Source: CAD feature listing. Evaluate the final solid. Frame: model axes, mm. Coordinates: 2 decimals unless noted, no trailing zeros. Order: outer loops, then holes, each group sorted by start corner. A loop starts at its lowest first (then second) coordinate and runs counter-clockwise, first axis right, second up.
```python
from build123d import *

# Parameters (mm, degrees)
SKETCH_1_R      = 20
EXTRUDE_1_DEPTH = 44.4
SKETCH_2_W      = 2.53960462
SKETCH_2_H      = 1.7


with BuildPart() as part:
    # 草图1 → 凸台-拉伸1 (new body)
    with BuildSketch(Plane(origin=(0, 0, 0), x_dir=(1, 0, 0), z_dir=(0, 1, 0))):
        with Locations(Location((0, 0, 0), (0, 0, 270))):
            Circle(SKETCH_1_R)
    extrude(amount=EXTRUDE_1_DEPTH)

    # 草图2 → 切除-旋转1 (revolve, cut)
    with BuildSketch(Plane.XY, mode=Mode.PRIVATE) as cut_revolve_1_sk:
        with Locations((-20.01980231, 3.85)):
            Rectangle(SKETCH_2_W, SKETCH_2_H)
    cut_revolve_1 = revolve(cut_revolve_1_sk.sketch.rotate(Axis((0, 44.4, 0), (0, -1, 0)), 270), axis=Axis((0, 44.4, 0), (0, -1, 0)), mode=Mode.SUBTRACT)

    # 镜向1: 切除-旋转1 across plane
    add(cut_revolve_1.mirror(Plane(origin=(0, 22.2, 0), x_dir=(0, 0, 1), z_dir=(0, -1, 0))), mode=Mode.SUBTRACT)


solid = part.part
```
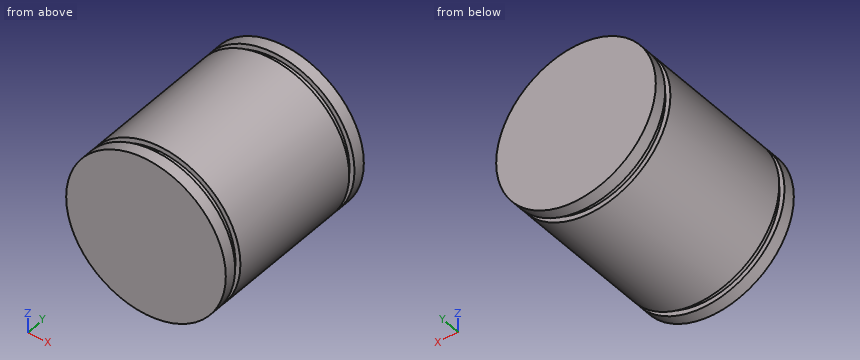
1. Contact query for flat-ended pins moving along their axis: P1, Ø2, axis at y = 39, z = 10.5, coming from the +X side; P2, Ø12, axis at y = 28.5, z = -8.5, coming from the +X side; P3, Ø1, axis at y = 36, z = 16, coming from the +X side. Output: stop coordinate, or through.
2. Section query C-C, the plane z = 14. Output: boundary loops of the cut face in (x, y).
3. Section query B-B, the plane y = 26. Output: boundary loops of the cut face in (x, z), plus the area to 3 significant figures.
4. Section query A-A, the plane x = -6. Output: boundary loops of the cut face in (y, z).
5. Material intervals for line 1 along X through (y, z) = (5, 14.5); line 2 along Z through (x, y) = (-12, 24.5); line 3 along Z through (x, y) = (-2.5, 12), sorted ascending.
Answer key:
1. P1: stops at x = 17.6
1. P2: stops at x = 19.84
1. P3: stops at x = 12.64
2. outline: (-14.28, 0) - (14.28, 0) - (14.28, 3) - (12.47, 3) - (12.47, 4.7) - (14.28, 4.7) - (14.28, 39.7) - (12.47, 39.7) - (12.47, 41.4) - (14.28, 41.4) - (14.28, 44.4) - (-14.28, 44.4) - (-14.28, 41.4) - (-12.47, 41.4) - (-12.47, 39.7) - (-14.28, 39.7) - (-14.28, 4.7) - (-12.47, 4.7) - (-12.47, 3) - (-14.28, 3) - close
3. outline: circle Ø40 at (0, 0)
3. area: 1,260 mm2
4. outline: (0, -19.08) - (3, -19.08) - (3, -17.76) - (4.7, -17.76) - (4.7, -19.08) - (39.7, -19.08) - (39.7, -17.76) - (41.4, -17.76) - (41.4, -19.08) - (44.4, -19.08) - (44.4, 19.08) - (41.4, 19.08) - (41.4, 17.76) - (39.7, 17.76) - (39.7, 19.08) - (4.7, 19.08) - (4.7, 17.76) - (3, 17.76) - (3, 19.08) - (0, 19.08) - close
5. line 1: x = -13.77 to 13.77
5. line 2: z = -16 to 16
5. line 3: z = -19.84 to 19.84
